Design review of the part built by this model. Coordinates are the model's own, in mm. Coordinates: 2 decimals unless noted, no trailing zeros. Write each loop counter-clockwise with the first axis right and the second up, starting at its lowest first coordinate (ties: lowest second). Pieces come first, ordered by that corner, then holes. Notation, with made-up numbers: (78.5, -4.5) - (108.5, -4.5) arc R10 cw to (108.5, 3.5) - close; hole circle Ø10 at (57, -11). An arc over 180 degrees is marked (long way). Answer as CSV lines item,"result". Start each with the question number.
Q1. For line 1 along Y through (x, z) = (0, -1.25); line 2 along X through (y, z) = (412, 6.5); line 3 along Y through (x, z) = (94.5, -0.25), list the stretches that pass through material, from the lowest coordinate up. Write a range as [from, to].
Q2. Mouldability with a two-part tool opening along Y and no side actions: class faces 1 (the face through (4, 0, 0)), 2 (the face through (-263.025, 433.39, 0.112)), 3 (the face through (155, 398.8, -0.1)) as pulls with the +Y half, pulls with the -Y half, needs draft (parallel to the pull), parting line crosses it, or undercut.
Q3. Clearance check with a flat-ended pin moving along its axis: pin 1 (1 mm diameter, centred on y = 341.5, z = -0.5, fed in from -X). State where the tip first meets the part, or that it passes through.
Q4. We need section B-B (y = 350). Write out the cut boundary in (x, z).
Q5. We need section C-C (z = -3.75). Write out the cut boundary in (x, y), plus the area to 3 significant figures.
Q6. We need section A-A (x = 0). Write out the cut boundary in (y, z).
Q7. We need section D-D (x = 242). Write out the cut boundary in (y, z), plus the area to 3 significant figures.
from build123d import *

# Parameters (mm, degrees)
SKETCH1_R           = 162.5
BOSS_EXTRUDE1_DEPTH = 8


with BuildPart() as part:
    # Sketch1 → Boss-Extrude1 (new, symmetric)
    with BuildSketch(Plane.XY):
        Polygon((-225, 550), (225, 550), (300, 320), (300, 0), (-300, 0), (-300, 320), align=None)
        with Locations((0, 350)):
            Circle(SKETCH1_R, mode=Mode.SUBTRACT)
    extrude(amount=BOSS_EXTRUDE1_DEPTH, both=True)


solid = part.part
Results list:
1,line 1,"y = [0, 187.5], [512.5, 550]"
1,line 2,"x = [-270, -150.21], [150.21, 270]"
1,line 3,"y = [0, 217.8], [482.2, 550]"
2,face 1,"pulls with the -Y half"
2,face 2,"pulls with the +Y half"
2,face 3,"undercut"
3,pin 1,"stops at x = -293.15"
4,outline,"(-290.22, -8) - (-162.5, -8) - (-162.5, 8) - (-290.22, 8) - close; (162.5, -8) - (290.22, -8) - (290.22, 8) - (162.5, 8) - close"
5,outline,"(-300, 0) - (300, 0) - (300, 320) - (225, 550) - (-225, 550) - (-300, 320) - close; hole circle Ø325 at (0, 350)"
5,area,"230,000 mm2"
6,outline,"(0, -8) - (187.5, -8) - (187.5, 8) - (0, 8) - close; (512.5, -8) - (550, -8) - (550, 8) - (512.5, 8) - close"
7,outline,"(0, -8) - (497.87, -8) - (497.87, 8) - (0, 8) - close"
7,area,"7,970 mm2"
